The drawing under review shows one solid part. Ordinate dimensions are in mm from its lowest x, y, z. Give positions to 0.01 mm unless a question says otherwise; leave off trailing zeros. Order: outer loops, then holes, each group sorted by start corner. A loop starts at its lowest first (then second) coordinate and runs counter-clockwise, first axis right, second up. Notation, with made-up numbers: (-40, 61) - (-24, 61) arc R5 cw to (-24, 65) - close; hole circle Ø5 at (73.25, 35.25). An arc over 180 degrees is marked (long way). Use CSV: the item, a comma, the result in double quotes. Start each with the question number.
1. Take a section at B-B, the plane y = 20. State the section outline as (x, z) points.
2. For pin 1 (10 mm diameter, centred on x = 26, y = 24.5, fed in from -Z), flat-tipped, find the tip position at first contact; note if it passes through.
3. To check wall thickness, follow line 1 (X direction, y = 20, z = 1.75); line 2 (X direction, y = 22, z = 2.25); line 3 (Y direction, x = 123, z = 4.25). State the ranges of each line that lie inside material, in increasing order. Write a range as [from, to].
4. Take a section at A-A, the plane x = 123. State the section outline as (y, z) points.
5. Take a section at C-C, the plane z = 5.25. State the section outline as (x, y) points.
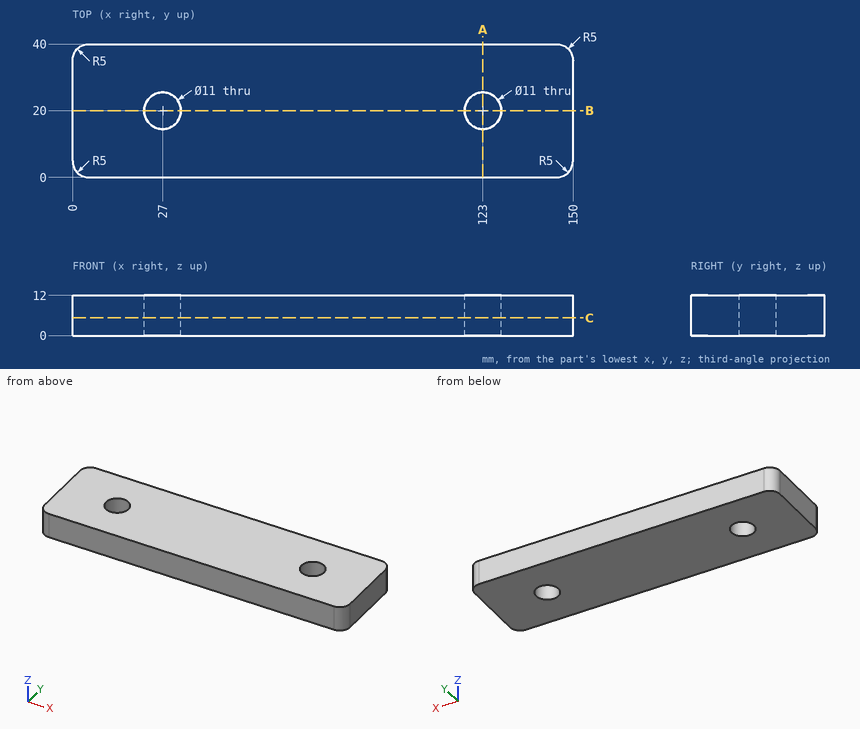
Determined:
1,outline,"(0, 0) - (21.5, 0) - (21.5, 12) - (0, 12) - close; (32.5, 0) - (117.5, 0) - (117.5, 12) - (32.5, 12) - close; (128.5, 0) - (150, 0) - (150, 12) - (128.5, 12) - close"
2,pin 1,"stops at z = 0"
3,line 1,"x = [0, 21.5], [32.5, 117.5], [128.5, 150]"
3,line 2,"x = [0, 21.88], [32.12, 117.88], [128.12, 150]"
3,line 3,"y = [0, 14.5], [25.5, 40]"
4,outline,"(0, 0) - (14.5, 0) - (14.5, 12) - (0, 12) - close; (25.5, 0) - (40, 0) - (40, 12) - (25.5, 12) - close"
5,outline,"(0, 5) arc R5 ccw to (5, 0) - (145, 0) arc R5 ccw to (150, 5) - (150, 35) arc R5 ccw to (145, 40) - (5, 40) arc R5 ccw to (0, 35) - close; hole circle Ø11 at (27, 20); hole circle Ø11 at (123, 20)"
